from build123d import *

# Parameters (mm, degrees)
CUT_EXTRUDE_1_REACH     = 194.094
SKETCH_2_W              = 3.96969722
SKETCH_2_H              = 10
HOLE_WIZARD_M10_2_D     = 8.5
HOLE_WIZARD_M10_2_DEPTH = 24.5
HOLE_WIZARD_M10_2_TIP   = 2.553657631


with BuildPart() as part:
    # 草图1 → 旋转1 (revolve)
    with BuildSketch(Plane.XY, mode=Mode.PRIVATE) as revolve_1_sk:
        Polygon((0, 77.5), (0, 19), (90, 19), (90, 65), (115, 65), (115, 90), (135, 90), (135, 120), (131, 120), (124.858175439, 104), (118.891690903, 104), (114, 120), (111, 120), (104.858175439, 104), (98.891690903, 104), (94, 120), (90, 120), (90, 115), (86, 115), (79.858175439, 99), (73.891690903, 99), (69, 115), (66, 115), (61.108309097, 99), (55.141824561, 99), (49, 115), (45, 115), (45, 77.5), (41, 77.5), (36.108309097, 61.5), (28.891690903, 61.5), (24, 77.5), (21, 77.5), (16.108309097, 61.5), (8.891690903, 61.5), (4, 77.5), align=None)
    revolve(revolve_1_sk.sketch.rotate(Axis((0, 0, 0), (1, 0, 0)), 90), axis=Axis((0, 0, 0), (1, 0, 0)))

    # 草图2 → 切除-拉伸1 (cut, up to next)
    with BuildSketch(Plane(origin=(90, 0, 0), x_dir=(0, 0, -1), z_dir=(1, 0, 0)), mode=Mode.PRIVATE) as cut_extrude_1_sk1:
        with Locations((-20.31515139, 0)):
            Rectangle(SKETCH_2_W, SKETCH_2_H)
    cut_extrude_1_tool1 = extrude(cut_extrude_1_sk1.sketch, amount=-CUT_EXTRUDE_1_REACH, mode=Mode.PRIVATE) & part.part
    add(cut_extrude_1_tool1.solids().sort_by_distance((90, 0, 20.315151))[0], mode=Mode.SUBTRACT)

    # M10 螺纹孔2
    with Locations(Plane(origin=(90, 0, 0), x_dir=(0, 0, -1), z_dir=(1, 0, 0))):
        with Locations((0, 42.5), (0, -42.5)):
            Hole(HOLE_WIZARD_M10_2_D / 2, depth=HOLE_WIZARD_M10_2_DEPTH)
            with Locations((0, 0, -(HOLE_WIZARD_M10_2_DEPTH + HOLE_WIZARD_M10_2_TIP / 2))):  # 118° drill point
                Cone(0, HOLE_WIZARD_M10_2_D / 2, HOLE_WIZARD_M10_2_TIP, mode=Mode.SUBTRACT)


solid = part.part
The listing builds one solid part. Answer for the finished solid, in the listing's coordinates (mm). A direction names the side the tool comes from. Coordinates: 2 decimals unless noted, no trailing zeros.
1) Find the intervals of material crossed by L1, parallel to Y at x = 76.5, z = 0; L2, parallel to Y at x = 103, z = 0; L3, parallel to X at y = 85, z = 65, in increasing order.
2) Flat-ended cylindrical pins translate along their axes: pin 1 Ø5 at (y, z) = (-25, 27) entering from +X; pin 2 Ø8 at (x, y) = (26, -56.5) entering from -Z; pin 3 Ø4.5 at (x, z) = (65, 21) entering from -Y. Find the tip coordinate at first contact, or state that the pin passes through.
3) Find section A-A on y = 70. Give the number of separate pieces and of enclosed holes in the cut face, then the cut area to 3 significant figures.
4) A tool of negligible diameter and unlimited length cuts with its end or side. For faces 1 (the face through (91.972, -101.184, 64.511)), 2 (the face through (42.972, 68.756, 35.762)), 3 (the face through (135, -89, -17)), 4 (the face through (115, 60, -26)), 5 (the face through (105.16, -103.89, -13.64)), from which of +Z, -Z, +X, -X, +Y, -Y can it reach the whole face along a straight path? Write none if from no direction.
5) Determine the mould class of faces 6 (the face through (63.39, 41.845, -0.341)), 7 (the face through (22.479, 68.756, 35.762)), 8 (the face through (0, 16, 16)) for opening direction Z: pulls with the +Z half, pulls with the -Z half, needs draft (parallel to the pull), parting line crosses it, or undercut.
Values:
1. L1: y = -99 to -46.75, -38.25 to -19, 19 to 38.25, 46.75 to 99
1. L2: y = -104 to -65, 65 to 104
1. L3: x = 45 to 52.07, 63.56 to 71.44, 82.93 to 97.97, 106.01 to 117.97, 126.01 to 135
2. pin 1: stops at x = 90
2. pin 2: stops at z = -56.51
2. pin 3: stops at y = -113.42
3. separate pieces: 3
3. enclosed holes: 0
3. area: 14,000 mm2
4. face 1: +X, -X
4. face 2: -X
4. face 3: +Z, -Z, +X, +Y, -Y
4. face 4: +X
4. face 5: none
5. face 6: undercut
5. face 7: parting line crosses it
5. face 8: needs draft
